from build123d import *

# Parameters (mm, degrees)
SKETCH_2_R          = 40
EXTRUDE_1_DEPTH     = 60
SKETCH_1_R          = 19.5
CUT_EXTRUDE_1_DEPTH = 40
CUT_EXTRUDE_START   = -15
CUT_EXTRUDE_2_DEPTH = 15
SKETCH_4_W          = 20
SKETCH_4_H          = 7.082368082
CUT_EXTRUDE_3_DEPTH = 30


with BuildPart() as part:
    # 草图2 → 凸台-拉伸1 (new body)
    with BuildSketch(Plane.XY):
        Circle(SKETCH_2_R)
    extrude(amount=EXTRUDE_1_DEPTH)

    # 草图1 → 切除-拉伸1 (cut)
    with BuildSketch(Plane.XY):
        Circle(SKETCH_1_R)
    extrude(amount=CUT_EXTRUDE_1_DEPTH, mode=Mode.SUBTRACT)

    # 草图3 → 切除-拉伸2 (cut)
    with BuildSketch(Plane.XY.offset(60).offset(CUT_EXTRUDE_START)):
        with BuildLine():
            Line((22.230762114, 21.495190528), (29.730762114, 8.504809472))
            Line((29.730762114, 8.504809472), (37.776643972, 13.150101528))
            ThreePointArc((37.776643972, 13.150101528), (34.641016151, 20), (30.276643972, 26.140482585))
            Line((30.276643972, 26.140482585), (22.230762114, 21.495190528))
        make_face()
        with BuildLine():
            Line((-7.5, 39.290584114), (-7.5, 30))
            Line((-7.5, 30), (7.5, 30))
            Line((7.5, 30), (7.5, 39.290584114))
            ThreePointArc((7.5, 39.290584114), (0, 40), (-7.5, 39.290584114))
        make_face()
        with BuildLine():
            Line((29.730762114, -8.504809472), (22.230762114, -21.495190528))
            Line((22.230762114, -21.495190528), (30.276643972, -26.140482585))
            ThreePointArc((30.276643972, -26.140482585), (34.641016151, -20), (37.776643972, -13.150101528))
            Line((37.776643972, -13.150101528), (29.730762114, -8.504809472))
        make_face()
        with BuildLine():
            Line((7.5, -30), (-7.5, -30))
            Line((-7.5, -30), (-7.5, -39.290584114))
            ThreePointArc((-7.5, -39.290584114), (0, -40), (7.5, -39.290584114))
            Line((7.5, -39.290584114), (7.5, -30))
        make_face()
        with BuildLine():
            Line((-22.230762114, -21.495190528), (-29.730762114, -8.504809472))
            Line((-29.730762114, -8.504809472), (-37.776643972, -13.150101528))
            ThreePointArc((-37.776643972, -13.150101528), (-34.641016151, -20), (-30.276643972, -26.140482585))
            Line((-30.276643972, -26.140482585), (-22.230762114, -21.495190528))
        make_face()
        with BuildLine():
            Line((-29.730762114, 8.504809472), (-22.230762114, 21.495190528))
            Line((-22.230762114, 21.495190528), (-30.276643972, 26.140482585))
            ThreePointArc((-30.276643972, 26.140482585), (-34.641016151, 20), (-37.776643972, 13.150101528))
            Line((-37.776643972, 13.150101528), (-29.730762114, 8.504809472))
        make_face()
    extrude(amount=CUT_EXTRUDE_2_DEPTH, mode=Mode.SUBTRACT)

    # 草图4 → 切除-拉伸3 (cut)
    with BuildSketch(Plane(origin=(0, 0, 0), x_dir=(-1, 0, 0), z_dir=(0, 0, -1))):
        with Locations((0, 19.458815959)):
            Rectangle(SKETCH_4_W, SKETCH_4_H)
    extrude(amount=-CUT_EXTRUDE_3_DEPTH, mode=Mode.SUBTRACT)


solid = part.part
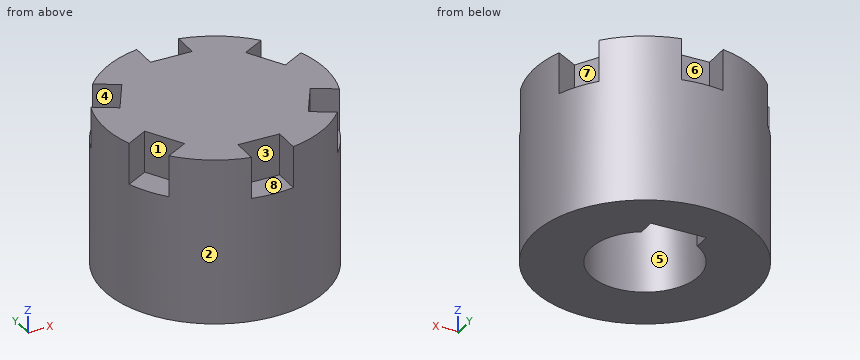
Verification items for the finished model (mm, model axes). Face numbers are marked on the shaded views. A direction names the side the tool comes from. Coordinates: 2 decimals unless noted, no trailing zeros. Order: outer loops, then holes, each group sorted by start corner. A loop starts at its lowest first (then second) coordinate and runs counter-clockwise, first axis right, second up.
1. Sectioned sample at C-C, the plane x = 0. Record the cut outline in (y, z).
Results found:
outline: (-40, 0) - (-19.5, 0) - (-19.5, 40) - (19.5, 40) - (19.5, 30) - (23, 30) - (23, 0) - (40, 0) - (40, 45) - (30, 45) - (30, 60) - (-30, 60) - (-30, 45) - (-40, 45) - close
2. Go/stop test with flat-tipped pins: pin 1 Ø4.5 at (y, z) = (-33.5, 53) entering from +X; pin 2 Ø1.5 at (x, z) = (-17, 35) entering from +Y; pin 3 Ø8 at (y, z) = (10.5, 53) entering from +X. Record where each tip stops, or that it passes through.
Results found:
pin 1: stops at x = 24.97
pin 2: stops at y = 36.55
pin 3: stops at x = 39.47
3. Scan lines: line 1 (Y direction, x = 27, z = 52.5); line 2 (Y direction, x = 0, z = 9); line 3 (X direction, y = 0, z = 20.5). Record each from-to range of solid material in increasing order.
Results found:
line 1: y = -29.51 to -24.25, -13.23 to 13.23, 24.25 to 29.51
line 2: y = -40 to -19.5, 23 to 40
line 3: x = -40 to -19.5, 19.5 to 40
4. Sectioned sample at D-D, the plane y = 0. Record the cut outline in (x, z).
Results found:
outline: (-40, 0) - (-19.5, 0) - (-19.5, 40) - (19.5, 40) - (19.5, 0) - (40, 0) - (40, 60) - (-40, 60) - close
5. Sectioned sample at B-B, the plane z = 54.5. Record the cut outline in (x, y), and give its area (3 significant figures).
Results found:
outline: (-37.78, -13.15) - (-29.73, -8.5) - (-22.23, -21.5) - (-30.28, -26.14) arc R40 ccw to (-7.5, -39.29) - (-7.5, -30) - (7.5, -30) - (7.5, -39.29) arc R40 ccw to (30.28, -26.14) - (22.23, -21.5) - (29.73, -8.5) - (37.78, -13.15) arc R40 ccw to (37.78, 13.15) - (29.73, 8.5) - (22.23, 21.5) - (30.28, 26.14) arc R40 ccw to (7.5, 39.29) - (7.5, 30) - (-7.5, 30) - (-7.5, 39.29) arc R40 ccw to (-30.28, 26.14) - (-22.23, 21.5) - (-29.73, 8.5) - (-37.78, 13.15) arc R40 ccw to start
area: 4,150 mm2
6. Set-up check for the marked faces 1, 2, 3, 4 and 5: record each of +Z, -Z, +X, -X, +Y, -Y from which the full face is reachable in a straight line by a thin tool's end or side.
Results found:
face 1: +Z
face 2: +Z, -Z
face 3: +Z, -Y
face 4: +Z, -X
face 5: -Z
7. Release check for a two-part mould opening along Y. For the marked faces 6, 7 and 8 record: +Y half, -Y half, draft (parallel to the pull), parting line (faces both ways), or undercut.
Results found:
face 6: +Y half
face 7: undercut
face 8: draft
8. Sectioned sample at A-A, the plane z = 14. Record the cut outline in (x, y), and give its area (3 significant figures).
Results found:
outline: circle Ø80 at (0, 0); hole (-10, 16.74) arc R19.5 ccw (long way) to (10, 16.74) - (10, 23) - (-10, 23) - close
area: 3,740 mm2
